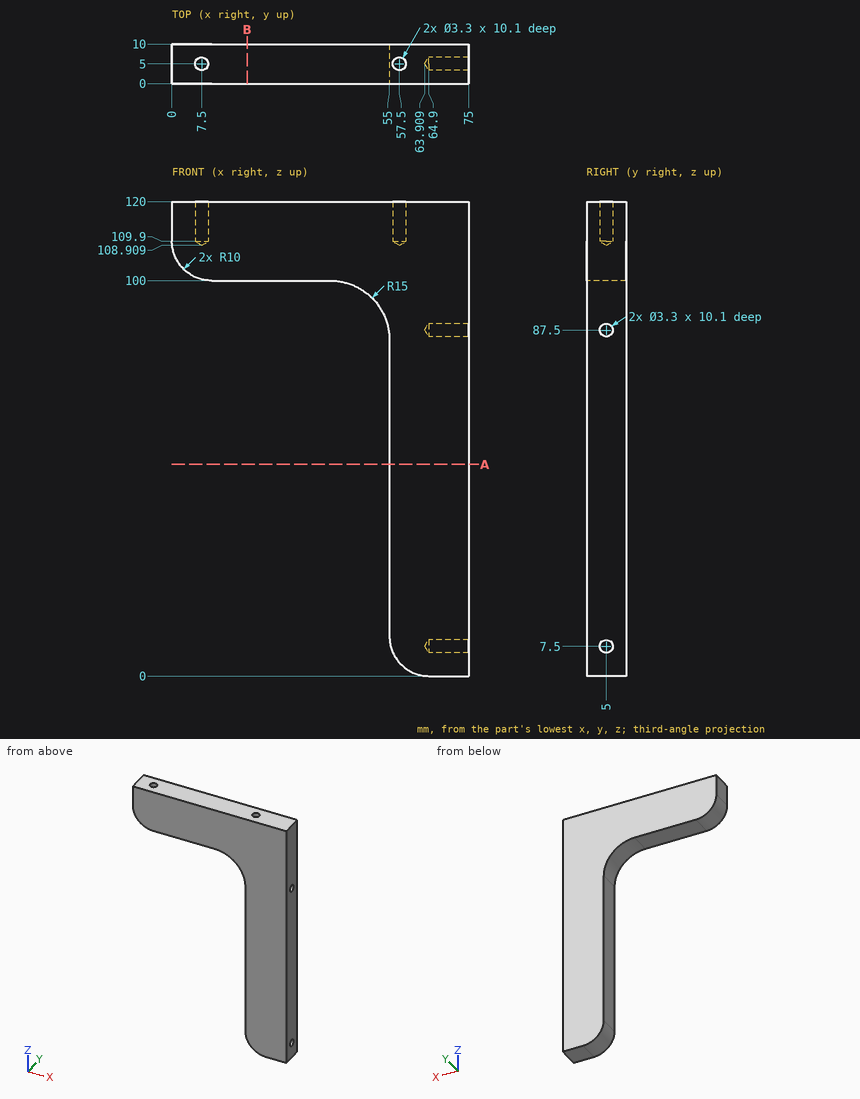
Check sheet for the drawn part. Datum: minimum x, y, z corner. Units: mm. Round coordinates to 2 decimals unless told otherwise and drop trailing zeros. Write each loop counter-clockwise with the first axis right and the second up, starting at its lowest first coordinate (ties: lowest second). Pieces come first, ordered by that corner, then holes. Notation, with made-up numbers: (40.25, 34.5) -> (63.25, 34.5) arc R21 ccw to (63.25, 68.5) -> close; hole circle Ø4 at (20, 21.25). An arc over 180 degrees is marked (long way). Put each result on its own line as item: value.
(1) Material ranges on line 1 (Z direction, x = 67.75, y = 5); line 2 (X direction, y = 5, z = 113.5); line 3 (Y direction, x = 57.5, z = 117.5), recorded low to high.
Values found:
line 1: z = 0 to 5.85, 9.15 to 85.85, 89.15 to 120
line 2: x = 0 to 5.85, 9.15 to 55.85, 59.15 to 75
line 3: y = 0 to 3.35, 6.65 to 10
(2) Sectioned sample at B-B (x = 19). Enter the section's corners in (y, z).
Values found:
outline: (0, 100) -> (10, 100) -> (10, 120) -> (0, 120) -> close
(3) Go/stop test with flat-tipped pins: pin 1 Ø2 at (y, z) = (5, 87.5) entering from -X; pin 2 Ø3 at (y, z) = (5.5, 46) entering from -X; pin 3 Ø2 at (x, y) = (33, 4.5) entering from -Z. Record where each tip stops, or that it passes through.
Values found:
pin 1: stops at x = 54.59
pin 2: stops at x = 55
pin 3: stops at z = 100
(4) Sectioned sample at A-A (z = 53.5). Enter the section's corners in (x, y).
Values found:
outline: (55, 0) -> (75, 0) -> (75, 10) -> (55, 10) -> close
